Geometry check sheet. Reference: the model listing, model coordinates, mm. A direction names the side the tool comes from. Coordinates: 2 decimals unless noted, no trailing zeros. Write each loop counter-clockwise with the first axis right and the second up, starting at its lowest first coordinate (ties: lowest second). Pieces come first, ordered by that corner, then holes. Notation, with made-up numbers: (60.25, 25) -> (115.25, 25) arc R33 cw to (115.25, 63) -> close; hole circle Ø1 at (7.25, 19). An arc over 180 degrees is marked (long way). Answer as CSV lines item,"result".
```python
from build123d import *

# Parameters (mm, degrees)
F_30X20X2_5_1_DEPTH = 568
CUT_EXTRUDE_1_REACH = 570.55
SKETCH_6_R          = 10.5
HOLE_WIZARD_M8_1_D  = 10
HOLE_WIZARD_M5_1_D  = 4.2


with BuildPart() as part:
    # Sketch14 → 矩型管 30X20X2.5(1) (new body)
    with BuildSketch(Plane(origin=(0, 0, 0), x_dir=(-1, 0, 0), z_dir=(0, 1, 0))):
        with BuildLine():
            Line((-5, -15), (5, -15))
            ThreePointArc((5, -15), (8.535533906, -13.535533906), (10, -10))
            Line((10, -10), (10, 10))
            ThreePointArc((10, 10), (8.535533906, 13.535533906), (5, 15))
            Line((5, 15), (-5, 15))
            ThreePointArc((-5, 15), (-8.535533906, 13.535533906), (-10, 10))
            Line((-10, 10), (-10, -10))
            ThreePointArc((-10, -10), (-8.535533906, -13.535533906), (-5, -15))
        make_face()
        with BuildLine():
            Line((-5, -12.5), (5, -12.5))
            ThreePointArc((5, -12.5), (6.767766953, -11.767766953), (7.5, -10))
            Line((7.5, -10), (7.5, 10))
            ThreePointArc((7.5, 10), (6.767766953, 11.767766953), (5, 12.5))
            Line((5, 12.5), (-5, 12.5))
            ThreePointArc((-5, 12.5), (-6.767766953, 11.767766953), (-7.5, 10))
            Line((-7.5, 10), (-7.5, -10))
            ThreePointArc((-7.5, -10), (-6.767766953, -11.767766953), (-5, -12.5))
        make_face(mode=Mode.SUBTRACT)
    extrude(amount=F_30X20X2_5_1_DEPTH)

    # 草图6 → 切除-拉伸1 (cut, up to next)
    with BuildSketch(Plane.ZY.offset(10), mode=Mode.PRIVATE) as cut_extrude_1_sk1:
        with Locations(Location((0, 18.5, 0), (0, 0, 17.752790162))):
            Circle(SKETCH_6_R)
    cut_extrude_1_tool1 = extrude(cut_extrude_1_sk1.sketch, amount=-CUT_EXTRUDE_1_REACH, mode=Mode.PRIVATE) & part.part
    add(cut_extrude_1_tool1.solids().sort_by_distance((-10, 18.5, 0))[0], mode=Mode.SUBTRACT)

    # M8 间隙孔1 (through all)
    with Locations(Plane.ZY.offset(10)):
        with Locations((0, 538), (0, 378), (0, 18.5)):
            Hole(HOLE_WIZARD_M8_1_D / 2)

    # M5 螺纹孔1 (through all)
    with Locations(Plane(origin=(10, 0, 0), x_dir=(0, 0, -1), z_dir=(1, 0, 0))):
        with Locations((0, 516.5), (0, 284), (0, 71.5), (0, 59), (0, 43)):
            Hole(HOLE_WIZARD_M5_1_D / 2)


solid = part.part
```
Item 1: Thickness scan on probe 1 along X at (y, z) = (499.5, 4.5); probe 2 along Z at (x, y) = (-2.25, 393.5); probe 3 along X at (y, z) = (436.5, -11). Record the ranges inside material, lowest first.
Responses:
probe 1,"x = -10 to -7.5, 7.5 to 10"
probe 2,"z = -15 to -12.5, 12.5 to 15"
probe 3,"x = -9.9 to -7.29, 7.29 to 9.9"
Item 2: Cross-section at B-B, the plane x = 0. Record the cut outline in (y, z).
Responses:
outline,"(0, -15) -> (568, -15) -> (568, -12.5) -> (0, -12.5) -> close; (0, 12.5) -> (568, 12.5) -> (568, 15) -> (0, 15) -> close"
Item 3: Set-up check for faces 1 (the flat face through (0, 280, -15)), 2 (the flat face through (-7.5, 6, 0)), 3 (the cylindrical face through (-8.743, 8.044, 0.958)): record each of +Z, -Z, +X, -X, +Y, -Y from which the full face is reachable in a straight line by a thin tool's end or side.
Responses:
face 1,"-Z, +X, -X, +Y, -Y"
face 2,"+Y, -Y"
face 3,"-X"
Item 4: Cross-section at A-A, the plane y = 378. Record the cut outline in (x, z).
Responses:
outline,"(-10, -10) arc R5 ccw to (-5, -15) -> (5, -15) arc R5 ccw to (10, -10) -> (10, -5) -> (7.5, -5) -> (7.5, -10) arc R2.5 cw to (5, -12.5) -> (-5, -12.5) arc R2.5 cw to (-7.5, -10) -> (-7.5, -5) -> (-10, -5) -> close; (-10, 5) -> (-7.5, 5) -> (-7.5, 10) arc R2.5 cw to (-5, 12.5) -> (5, 12.5) arc R2.5 cw to (7.5, 10) -> (7.5, 5) -> (10, 5) -> (10, 10) arc R5 ccw to (5, 15) -> (-5, 15) arc R5 ccw to (-10, 10) -> close"
Item 5: Depth check by flat-ended pin: pin 1 Ø4 at (y, z) = (516.5, 0) entering from +X; pin 2 Ø11.5 at (y, z) = (18.5, 0) entering from -X. Enter the tip coordinate at first touch or a pass-through.
Responses:
pin 1,"passes through"
pin 2,"stops at x = 7.5"
Item 6: Cross-section at C-C, the plane y = 448. Record the cut outline in (x, z).
Responses:
outline,"(-10, -10) arc R5 ccw to (-5, -15) -> (5, -15) arc R5 ccw to (10, -10) -> (10, 10) arc R5 ccw to (5, 15) -> (-5, 15) arc R5 ccw to (-10, 10) -> close; hole (-7.5, -10) arc R2.5 ccw to (-5, -12.5) -> (5, -12.5) arc R2.5 ccw to (7.5, -10) -> (7.5, 10) arc R2.5 ccw to (5, 12.5) -> (-5, 12.5) arc R2.5 ccw to (-7.5, 10) -> close"
Item 7: Release check for a two-part mould opening along X. For faces 4 (the flat face through (7.5, 280, 0)), 5 (the cylindrical face through (8.768, 542.957, 0.651)), 6 (the flat face through (10, 280, 0)) record: +X half, -X half, draft (parallel to the pull), parting line (faces both ways), or undercut.
Responses:
face 4,"undercut"
face 5,"draft"
face 6,"+X half"
